```python
from build123d import *

# Parameters (mm, degrees)
SADDLE_BASE_BLOCK_DEPTH     = 30
THROUGH_HOLE_15_DEPTH       = 106.148704224
SLOT_CUT_DEPTH              = 15
CROSS_BOSS_PROFILE_SKETCH_R = 10
CROSS_BOSS_DEPTH            = 30
UPPER_PAD_SKETCH_W          = 20
UPPER_PAD_SKETCH_H          = 30
UPPER_PAD_DEPTH             = 15
NOTCH_CUT_DEPTH             = 30
NOTCH_FILL_BOSS_DEPTH       = 10


with BuildPart() as part:
    # Base Arch Profile Sketch → Saddle Base Block (new, symmetric)
    with BuildSketch(Plane.XY):
        with BuildLine():
            Line((20, -12.5), (50, -12.5))
            Line((50, -12.5), (50, 12.5))
            Line((50, 12.5), (-50, 12.5))
            Line((-50, 12.5), (-50, -12.5))
            Line((-50, -12.5), (-20, -12.5))
            ThreePointArc((-20, -12.5), (0, 7.5), (20, -12.5))
        make_face()
    extrude(amount=SADDLE_BASE_BLOCK_DEPTH, both=True)

    # Through Hole Sketch → Through Hole Ø15 (cut, through all)
    with BuildSketch(Plane.ZY.offset(50)):
        with BuildLine():
            Line((-15, -12.5), (15, -12.5))
            ThreePointArc((15, -12.5), (0, 2.5), (-15, -12.5))
        make_face()
    extrude(amount=-THROUGH_HOLE_15_DEPTH, mode=Mode.SUBTRACT)

    # Slot Profile Sketch → Slot Cut (cut)
    with BuildSketch(Plane.ZY.offset(50)):
        Polygon((0, 12.5), (10, 12.5), (10, 4.5), (-10, 4.5), (-10, 12.5), align=None)
    extrude(amount=-SLOT_CUT_DEPTH, mode=Mode.SUBTRACT)

    # Cross Boss Profile Sketch → Cross Boss (add)
    with BuildSketch(Plane(origin=(0, 12.5, 0), x_dir=(1, 0, 0), z_dir=(0, 1, 0))):
        Polygon((20, -10), (20, 10), (35, 10), (35, 20), (13, 20), (13, 15), (-13, 15), (-13, 20), (-35, 20), (-35, 10), (-20, 10), (-20, -10), (-35, -10), (-35, -20), (-13, -20), (-13, -15), (13, -15), (13, -20), (35, -20), (35, -10), align=None)
        with Locations(Location((0, 0, 0), (0, 0, 270))):
            Circle(CROSS_BOSS_PROFILE_SKETCH_R, mode=Mode.SUBTRACT)
    extrude(amount=CROSS_BOSS_DEPTH)

    # Upper Pad Sketch → Upper Pad (add)
    with BuildSketch(Plane.ZY.offset(20)):
        with Locations((0, 27.5)):
            Rectangle(UPPER_PAD_SKETCH_W, UPPER_PAD_SKETCH_H)
    extrude(amount=UPPER_PAD_DEPTH)

    # Notch Cut Sketch → Notch Cut (cut)
    with BuildSketch(Plane.XY.offset(20)):
        Polygon((-35, 12.5), (-13, 42.5), (-35, 42.5), align=None)
    extrude(amount=-NOTCH_CUT_DEPTH, mode=Mode.SUBTRACT)

    # Notch Fill Sketch → Notch Fill Boss (add)
    with BuildSketch(Plane.XY.offset(20)):
        Polygon((-35, 12.5), (-35, 42.5), (-13, 42.5), align=None)
    extrude(amount=-NOTCH_FILL_BOSS_DEPTH)


solid = part.part
```
For this review, take the finished solid that the model builds, in its own axes (mm). A direction names the side the tool comes from. Round coordinates to 2 decimals unless told otherwise and drop trailing zeros. Write each loop counter-clockwise with the first axis right and the second up, starting at its lowest first coordinate (ties: lowest second). Pieces come first, ordered by that corner, then holes. Notation, with made-up numbers: M 20.5,1 L 49.5,1 A20 ccw 49.5,5 Z; hole C -39.75,73.5 d2. An arc over 180 degrees is marked long. One line per item, written item: value. Start each with the question number.
(1) We need section A-A (z = 0). Give the boundary of the cut face in (x, y), and give its area (3 significant figures).
(2) The part is to be moulded in two halves that separate along X. For faces 1 (the flat face through (-35, 27, 15)), 2 (the flat face through (-43, 4.5, 0)), 3 (the flat face through (20, 27, 0)), 4 (the flat face through (-13, 27, 18)), say which applies: released by +X, released by -X, zero draft, split by the parting line, or undercut.
(3) Insertion check: pin 1 (12 mm diameter, centred on x = 28, y = 34.5, fed in from -Z); pin 2 (3 mm diameter, centred on y = 25.5, z = 7.5, fed in from -X); pin 3 (7.5 mm diameter, centred on x = -41.5, z = -1.5, fed in from +Y); pin 4 (10 mm diameter, centred on x = -31.5, y = 14, fed in from -Z). Each pin has a flat end and moves straight along its axis. Give the tip position at first contact, or say it passes through.
(4) Machinability: for faces 5 (the flat face through (-24, 28, 20)), 6 (the flat face through (0, 27, -15)), 7 (the cylindrical face through (-9.76, 27.29, -2.17)), 8 (the flat face through (24, 27, -20)), 9 (the flat face through (27, 27, -10)), which of the approach directions +Z, -Z, +X, -X, +Y, -Y give a long, thin tool a straight path to every point of the face, cutting with its end or side? Answer none if there is none.
(5) We need section C-C (x = 0). Give the boundary of the cut face in (y, z), and give its area (3 significant figures).
(6) Wall thickness on line 1 (Y direction, x = 0, z = -20.5); line 2 (Z direction, x = -3, y = 26.5); line 3 (X direction, y = 16, z = 16.5): over which ranges is each line inside the solid? List them lowest first.
(7) We need section D-D (y = 0.5). Give the boundary of the cut face in (x, z).
(8) We need section B-B (y = 17). Give the boundary of the cut face in (x, z), and give its area (3 significant figures).
Result:
1. outline: M -50,2.5 L -13.23,2.5 A20 cw 13.23,2.5 L 50,2.5 L 50,12.5 L 20,12.5 L 20,42.5 L 10,42.5 L 10,12.5 L -10,12.5 L -10,42.5 L -13,42.5 L -35,12.5 L -35,4.5 L -50,4.5 Z
1. area: 1,510 mm²
2. face 1: released by -X
2. face 2: zero draft
2. face 3: released by +X
2. face 4: undercut
3. pin 1: z = -20
3. pin 2: x = -26.57
3. pin 3: y = 4.5
3. pin 4: z = -30
4. face 5: +Z, +X, -X, +Y
4. face 6: -Z, +Y
4. face 7: +Y
4. face 8: -Z, +X, -X, +Y
4. face 9: +X, +Y
5. outline: M 7.5,-30 L 12.5,-30 L 12.5,-15 L 42.5,-15 L 42.5,-10 L 12.5,-10 L 12.5,10 L 42.5,10 L 42.5,15 L 12.5,15 L 12.5,30 L 7.5,30 Z
5. area: 600 mm²
6. line 1: 7.5 to 12.5
6. line 2: -15 to -9.54, 9.54 to 15
6. line 3: -35 to -13, 13 to 35
7. outline: M -50,-30 L -15.2,-30 L -15.2,-7.48 L -50,-7.48 Z; M -50,7.48 L -15.2,7.48 L -15.2,30 L -50,30 Z; M 15.2,-30 L 50,-30 L 50,-7.48 L 15.2,-7.48 Z; M 15.2,7.48 L 50,7.48 L 50,30 L 15.2,30 Z
8. outline: M -35,-20 L -13,-20 L -13,-15 L 13,-15 L 13,-20 L 35,-20 L 35,-10 L 20,-10 L 20,10 L 35,10 L 35,20 L 13,20 L 13,15 L -13,15 L -13,20 L -35,20 L -35,10 L -31.7,10 L -31.7,-10 L -35,-10 Z; hole C 0,0 d20
8. area: 1,860 mm²
